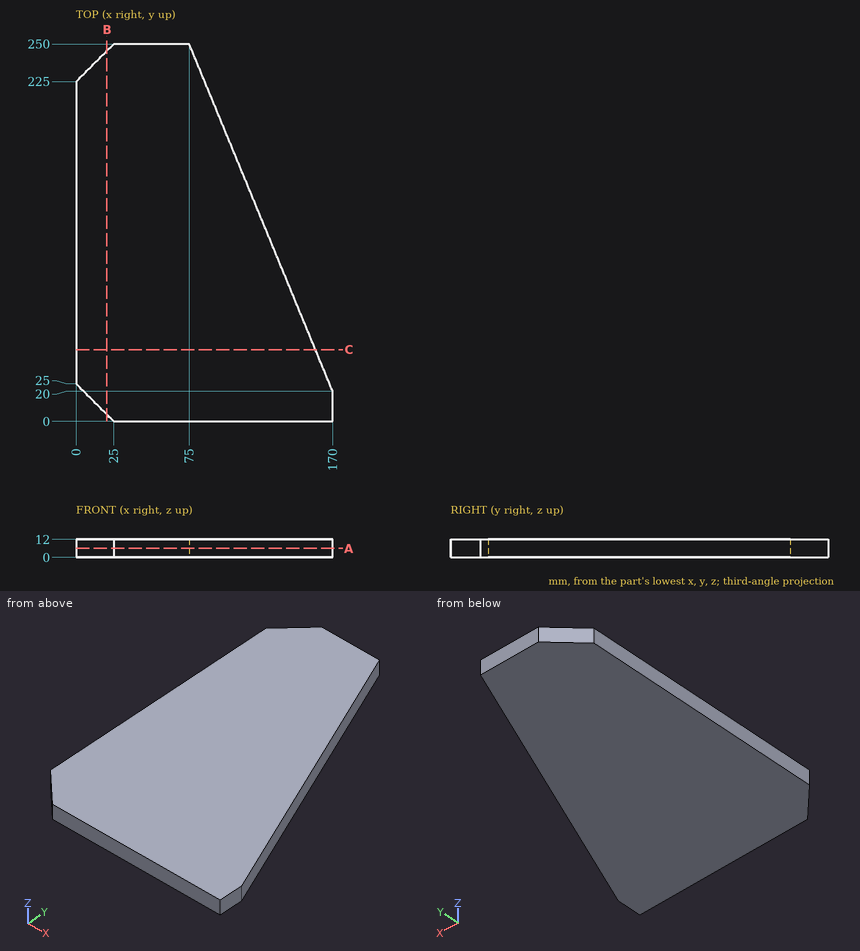
Part print with two shaded views. Sizes in mm from the minimum x, y, z corner. Round coordinates to 2 decimals unless told otherwise and drop trailing zeros. Order: outer loops, then holes, each group sorted by start corner. A loop starts at its lowest first (then second) coordinate and runs counter-clockwise, first axis right, second up. Notation, with made-up numbers: (35, -3) -> (65, -3) arc R29 ccw to (65, 29) -> close; hole circle Ø9 at (70, -32). An arc over 180 degrees is marked (long way). Use one line per item in the form item = value.
Item 1: Cut at B-B, the plane x = 20.5. Write the cut outline in (y, z).
Returned:
outline = (4.5, 0) -> (245.5, 0) -> (245.5, 12) -> (4.5, 12) -> close
Item 2: Drill centre lines: line 1 (X direction, y = 51.5, z = 2.25); line 2 (X direction, y = 58.5, z = 7.75); line 3 (Y direction, x = 83, z = 8). Where is each one in solid material? Low to high.
Returned:
line_1 = 0 to 156.99
line_2 = 0 to 154.1
line_3 = 0 to 230.63
Item 3: Cut at A-A, the plane z = 6. Write the cut outline in (x, y), and give its area (4 significant figures).
Returned:
outline = (0, 25) -> (25, 0) -> (170, 0) -> (170, 20) -> (75, 250) -> (25, 250) -> (0, 225) -> close
area = 30,950 mm^2
Item 4: Cut at C-C, the plane y = 47.5. Write the cut outline in (x, z).
Returned:
outline = (0, 0) -> (158.64, 0) -> (158.64, 12) -> (0, 12) -> close
